Geometry check sheet. Reference: the model listing, model coordinates, mm. A direction names the side the tool comes from. Round coordinates to 2 decimals unless told otherwise and drop trailing zeros. Write each loop counter-clockwise with the first axis right and the second up, starting at its lowest first coordinate (ties: lowest second). Pieces come first, ordered by that corner, then holes. Notation, with made-up numbers: (58, 9) - (93, 9) arc R9 cw to (93, 15) - close; hole circle Ø3 at (49, 68). An arc over 180 degrees is marked (long way). Return JSON: item names as keys, results as strings.
```python
from build123d import *

# Parameters (mm, degrees)
EXTRUDE_1_DEPTH = 12


with BuildPart() as part:
    # 草图2 → 凸台-拉伸1 (new body)
    with BuildSketch(Plane.ZY.offset(140.770328303)):
        with BuildLine():
            Line((-63, -168), (-63, -153))
            ThreePointArc((-63, -153), (-61.535533906, -149.464466094), (-58, -148))
            Line((-58, -148), (67, -148))
            Line((67, -148), (67, -68))
            Line((67, -68), (-58, -68))
            ThreePointArc((-58, -68), (-61.535533906, -66.535533906), (-63, -63))
            Line((-63, -63), (-63, -48))
            ThreePointArc((-63, -48), (-61.535533906, -44.464466094), (-58, -43))
            Line((-58, -43), (67, -43))
            Line((67, -43), (67, -8))
            Line((67, -8), (-98, -8))
            Line((-98, -8), (-98, -208))
            Line((-98, -208), (67, -208))
            Line((67, -208), (67, -173))
            Line((67, -173), (-58, -173))
            ThreePointArc((-58, -173), (-61.535533906, -171.535533906), (-63, -168))
        make_face()
    extrude(amount=EXTRUDE_1_DEPTH)


solid = part.part
```
(1) Material ranges on line 1 along Y through (x, z) = (-144, -3); line 2 along Y through (x, z) = (-148.5, -59.5); line 3 along Z through (x, y) = (-141.75, -158), recorded low to high. Write a range as [from, to].
Response values:
{"line 1": "y = [-208, -173], [-148, -68], [-43, -8]", "line 2": "y = [-208, -172.77], [-148.23, -67.77], [-43.23, -8]", "line 3": "z = [-98, -63]"}
(2) Access from +Z, -Z, +X, -X, +Y, -Y to the whole of each face (thin tool, end or side, straight path). Record for faces 5 (the face through (-147, -107, -98)), 6 (the face through (-147, -56, -63)).
Response values:
{"face 5": "-Z, +X, -X, +Y, -Y", "face 6": "+Z, +X, -X"}
(3) Gauge pin test, flat end, axial feed: pin 1 (6 mm diameter, centred on y = -63, z = -59, fed in from -X). Record the tip position at first contact, or that the pin passes through.
Response values:
{"pin 1": "passes through"}
(4) Section check C-C, the plane y = -58.5. Enter the section's corners in (x, z).
Response values:
{"outline": "(-152.77, -98) - (-140.77, -98) - (-140.77, -63) - (-152.77, -63) - close"}
(5) Release check for a two-part mould opening along Y. For faces 1 (the face through (-147, -26, 67)), 2 (the face through (-147, -8, -14)), 3 (the face through (-147, -208, -17)), 4 (the face through (-147, -173, 5)) record: pulls with the +Y half, pulls with the -Y half, needs draft (parallel to the pull), parting line crosses it, or undercut.
Response values:
{"face 1": "needs draft", "face 2": "pulls with the +Y half", "face 3": "pulls with the -Y half", "face 4": "undercut"}
(6) Section check B-B, the plane x = -149. Enter the section's corners in (y, z).
Response values:
{"outline": "(-208, -98) - (-8, -98) - (-8, 67) - (-43, 67) - (-43, -58) arc R5 cw to (-48, -63) - (-63, -63) arc R5 cw to (-68, -58) - (-68, 67) - (-148, 67) - (-148, -58) arc R5 cw to (-153, -63) - (-168, -63) arc R5 cw to (-173, -58) - (-173, 67) - (-208, 67) - close"}
(7) Section check A-A, the plane z = -10.5. Enter the section's corners in (x, y).
Response values:
{"outline": "(-152.77, -208) - (-140.77, -208) - (-140.77, -173) - (-152.77, -173) - close; (-152.77, -148) - (-140.77, -148) - (-140.77, -68) - (-152.77, -68) - close; (-152.77, -43) - (-140.77, -43) - (-140.77, -8) - (-152.77, -8) - close"}
